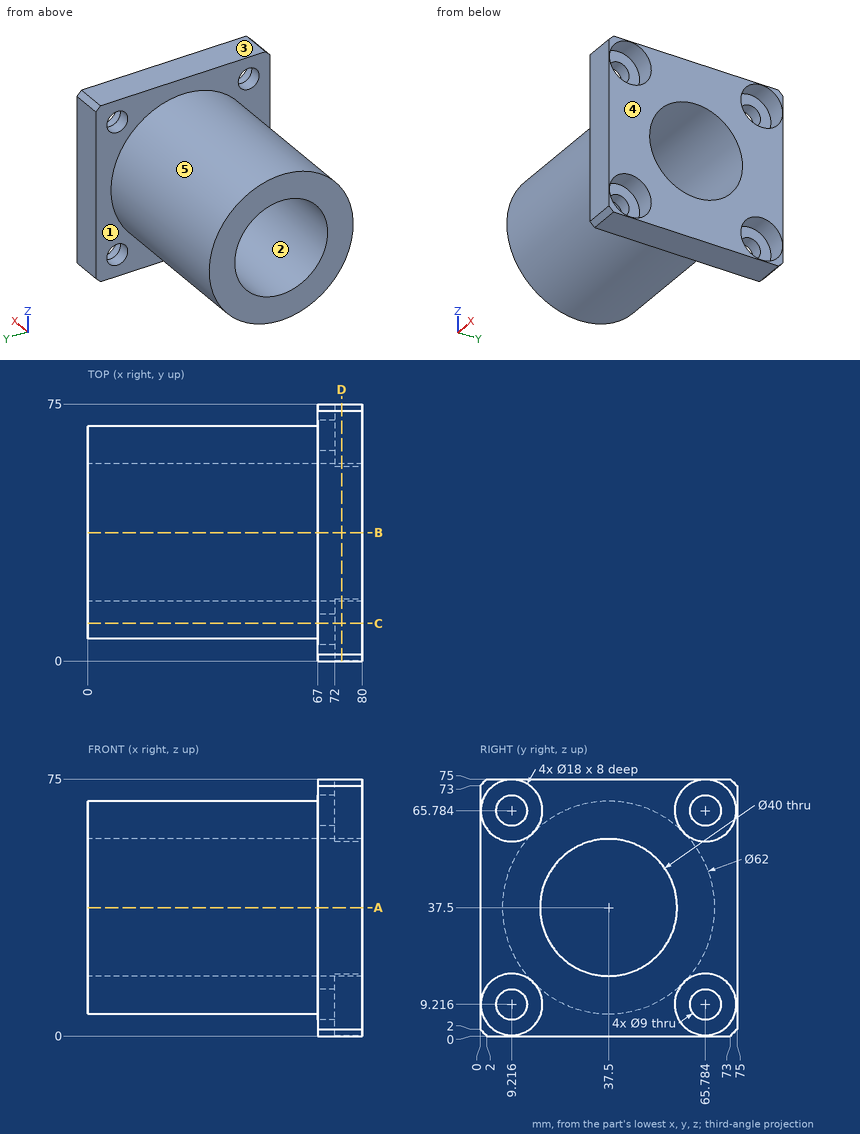
Drawing for the job (mm, zero at the part's lowest x, y, z). A direction names the side the tool comes from. Coordinates: 2 decimals unless noted, no trailing zeros. Write each loop counter-clockwise with the first axis right and the second up, starting at its lowest first coordinate (ties: lowest second). Pieces come first, ordered by that corner, then holes. Notation, with made-up numbers: (-36.75, 51) -> (-20.75, 51) arc R15 cw to (-20.75, 72) -> close; hole circle Ø9 at (36.5, -17.5). An arc over 180 degrees is marked (long way). One line per item, written item: value. Start each with the question number.
1) Slice it at D-D on x = 74. Write the cut outline in (y, z), then the cut area to 3 significant figures.
2) Probe probe 1 along X at (y, z) = (71, 28); probe 2 along Y at (x, z) = (46, 28); probe 3 along Y at (x, z) = (65.5, 26). List the from-to ranges inside material, lowest first.
3) Which spindle directions (+Z, -Z, +X, -X, +Y, -Y) get a long thin tool onto all of the face, cutting with end or side? Do the marked faces 4 and 5. Say none if no direction does.
4) Flat gauge pins, fed straight in: pin 1 Ø4 at (x, y) = (52, 45.5) entering from +Z; pin 2 Ø16 at (y, z) = (65.78, 9.22) entering from +X; pin 3 Ø3 at (x, y) = (10.5, 26.5) entering from -Z; pin 4 Ø5.5 at (y, z) = (65.78, 9.22) entering from -X. Where does each tip first touch, or does it go through?
5) Pull direction Z, two halves, no side cores. Call the marked faces 1, 2 and 3: +Z half, -Z half, draft (parallel to the pull), parting line (faces both ways), or undercut.
6) Slice it at C-C on y = 11. Count the separate pieces of the cut face and the enclosed holes in it, then the cut area to 3 significant figures.
7) Slice it at A-A on z = 37.5. Write the cut outline in (x, y), then the cut area to 3 significant figures.
Answers follow:
1. outline: (0, 2) -> (2, 0) -> (73, 0) -> (75, 2) -> (75, 73) -> (73, 75) -> (2, 75) -> (0, 73) -> close; hole circle Ø18 at (9.22, 9.22); hole circle Ø18 at (9.22, 65.78); hole circle Ø40 at (37.5, 37.5); hole circle Ø18 at (65.78, 9.22); hole circle Ø18 at (65.78, 65.78)
1. area: 3,340 mm2
2. probe 1: 67 to 80
2. probe 2: 7.99 to 19.9, 55.1 to 67.01
2. probe 3: 8.71 to 21.14, 53.86 to 66.29
3. face 4: +Z, -Z, +X, +Y, -Y
3. face 5: -X
4. pin 1: z = 67.91
4. pin 2: x = 72
4. pin 3: z = 7.99
4. pin 4: through
5. face 1: draft
5. face 2: undercut
5. face 3: +Z half
6. separate pieces: 3
6. enclosed holes: 0
6. area: 2,770 mm2
7. outline: (0, 6.5) -> (67, 6.5) -> (67, 0) -> (80, 0) -> (80, 17.5) -> (0, 17.5) -> close; (0, 57.5) -> (80, 57.5) -> (80, 75) -> (67, 75) -> (67, 68.5) -> (0, 68.5) -> close
7. area: 1,930 mm2
